from build123d import *

# Parameters (mm, degrees)
SKETCH_1_W             = 88
SKETCH_1_H             = 10
EXTRUDE_1_DEPTH        = 250
SKETCH_2_W             = 2
SKETCH_2_H             = 5
CUT_EXTRUDE_1_DEPTH    = 254.891709199
HOLE_WIZARD_M5_1_D     = 4.2
HOLE_WIZARD_M5_1_DEPTH = 10
HOLE_WIZARD_M5_1_TIP   = 1.2618073
HOLE_WIZARD_M5_2_D     = 4.2
HOLE_WIZARD_M5_2_DEPTH = 10
HOLE_WIZARD_M5_2_TIP   = 1.2618073
SKETCH_7_R             = 3.25
CUT_EXTRUDE_2_DEPTH    = 255.039367028
SKETCH_8_R             = 5.5
CUT_EXTRUDE_3_DEPTH    = 6
SKETCH_9_R             = 2.75
CUT_EXTRUDE_4_DEPTH    = 255.039367028
SKETCH_10_R            = 4.5
CUT_EXTRUDE_5_DEPTH    = 5


with BuildPart() as part:
    # 草图1 → 凸台-拉伸1 (new body)
    with BuildSketch(Plane.XY):
        Rectangle(SKETCH_1_W, SKETCH_1_H)
    extrude(amount=EXTRUDE_1_DEPTH)

    # 草图2 → 切除-拉伸1 (cut, through all)
    with BuildSketch(Plane.XY.offset(250)):
        with Locations((-41, 2.5)):
            Rectangle(SKETCH_2_W, SKETCH_2_H)
        with Locations((41, 2.5)):
            Rectangle(SKETCH_2_W, SKETCH_2_H)
    extrude(amount=-CUT_EXTRUDE_1_DEPTH, mode=Mode.SUBTRACT)

    # M5 螺纹孔1
    with Locations(Plane(origin=(-32, 0, 250), x_dir=(1, 0, 0), z_dir=(0, 0, 1))):
        with Locations((0, 0), (64, 0)):
            Hole(HOLE_WIZARD_M5_1_D / 2, depth=HOLE_WIZARD_M5_1_DEPTH)
            with Locations((0, 0, -(HOLE_WIZARD_M5_1_DEPTH + HOLE_WIZARD_M5_1_TIP / 2))):  # 118° drill point
                Cone(0, HOLE_WIZARD_M5_1_D / 2, HOLE_WIZARD_M5_1_TIP, mode=Mode.SUBTRACT)

    # M5 螺纹孔2
    with Locations(Plane(origin=(32, 0, 0), x_dir=(-1, 0, 0), z_dir=(0, 0, -1))):
        with Locations((0, 0), (64, 0)):
            Hole(HOLE_WIZARD_M5_2_D / 2, depth=HOLE_WIZARD_M5_2_DEPTH)
            with Locations((0, 0, -(HOLE_WIZARD_M5_2_DEPTH + HOLE_WIZARD_M5_2_TIP / 2))):  # 118° drill point
                Cone(0, HOLE_WIZARD_M5_2_D / 2, HOLE_WIZARD_M5_2_TIP, mode=Mode.SUBTRACT)

    # 草图7 → 切除-拉伸2 (cut, through all)
    with BuildSketch(Plane(origin=(0, 5, 0), x_dir=(1, 0, 0), z_dir=(0, 1, 0))):
        with Locations(Location((-15, -80, 0), (0, 0, 270))):
            Circle(SKETCH_7_R)
        with Locations(Location((15, -80, 0), (0, 0, 270))):
            Circle(SKETCH_7_R)
        with Locations(Location((15, -170, 0), (0, 0, 90))):
            Circle(SKETCH_7_R)
        with Locations(Location((-15, -170, 0), (0, 0, 90))):
            Circle(SKETCH_7_R)
    extrude(amount=-CUT_EXTRUDE_2_DEPTH, mode=Mode.SUBTRACT)

    # 草图8 → 切除-拉伸3 (cut)
    with BuildSketch(Plane(origin=(0, 5, 0), x_dir=(1, 0, 0), z_dir=(0, 1, 0))):
        with Locations(Location((-15, -80, 0), (0, 0, 270))):
            Circle(SKETCH_8_R)
        with Locations(Location((15, -80, 0), (0, 0, 270))):
            Circle(SKETCH_8_R)
        with Locations(Location((-15, -170, 0), (0, 0, 270))):
            Circle(SKETCH_8_R)
        with Locations(Location((15, -170, 0), (0, 0, 270))):
            Circle(SKETCH_8_R)
    extrude(amount=-CUT_EXTRUDE_3_DEPTH, mode=Mode.SUBTRACT)

    # 草图9 → 切除-拉伸4 (cut, through all)
    with BuildSketch(Plane.XZ.offset(5)):
        with Locations(Location((-32, 232, 0), (0, 0, 270))):
            Circle(SKETCH_9_R)
        with Locations(Location((-32, 202, 0), (0, 0, 270))):
            Circle(SKETCH_9_R)
    extrude(amount=-CUT_EXTRUDE_4_DEPTH, mode=Mode.SUBTRACT)

    # 草图10 → 切除-拉伸5 (cut)
    with BuildSketch(Plane.XZ.offset(5)):
        with Locations(Location((-32, 232, 0), (0, 0, 270))):
            Circle(SKETCH_10_R)
        with Locations(Location((-32, 202, 0), (0, 0, 270))):
            Circle(SKETCH_10_R)
    extrude(amount=-CUT_EXTRUDE_5_DEPTH, mode=Mode.SUBTRACT)


solid = part.part
Design review of the part built by this model. Coordinates are the model's own, in mm. A direction names the side the tool comes from. Round coordinates to 2 decimals unless told otherwise and drop trailing zeros. Order: outer loops, then holes, each group sorted by start corner. A loop starts at its lowest first (then second) coordinate and runs counter-clockwise, first axis right, second up.
1) Consider section B-B (z = 170). State the section outline as (x, y) points, plus the area to 3 significant figures.
The answers:
outline: (-44, -5) - (-18.25, -5) - (-18.25, -1) - (-20.5, -1) - (-20.5, 5) - (-40, 5) - (-40, 0) - (-42, 0) - (-42, 5) - (-44, 5) - close; (-11.75, -5) - (11.75, -5) - (11.75, -1) - (9.5, -1) - (9.5, 5) - (-9.5, 5) - (-9.5, -1) - (-11.75, -1) - close; (18.25, -5) - (44, -5) - (44, 5) - (42, 5) - (42, 0) - (40, 0) - (40, 5) - (20.5, 5) - (20.5, -1) - (18.25, -1) - close
area: 676 mm2
2) Draft analysis for pull direction Z (two halves, no side actions). For faces 1 (the conical face through (31.8, 0.31, 11.04)), 2 (the flat face through (-35, 0, 202)), 3 (the flat face through (-44, 0, 123)), state which applies: released by +Z, released by -Z, zero draft, split by the parting line, or undercut.
The answers:
face 1: released by -Z
face 2: undercut
face 3: zero draft
3) Clearance check with flat-ended pins moving along their axes: pin 1 Ø9 at (x, z) = (15, 79.5) entering from +Y; pin 2 Ø7 at (x, z) = (-32, 232) entering from -Y; pin 3 Ø4 at (x, y) = (-32, 0) entering from -Z. State where each tip first meets the part, or that it passes through.
The answers:
pin 1: stops at y = -1
pin 2: stops at y = 0
pin 3: stops at z = 10.06
4) Consider section A-A (x = -15). State the section outline as (y, z) points, plus the area to 3 significant figures.
The answers:
outline: (-5, 0) - (5, 0) - (5, 74.5) - (-1, 74.5) - (-1, 76.75) - (-5, 76.75) - close; (-5, 83.25) - (-1, 83.25) - (-1, 85.5) - (5, 85.5) - (5, 164.5) - (-1, 164.5) - (-1, 166.75) - (-5, 166.75) - close; (-5, 173.25) - (-1, 173.25) - (-1, 175.5) - (5, 175.5) - (5, 250) - (-5, 250) - close
area: 2,320 mm2
5) For L1, parallel to X at y = -4.2, z = 80; L2, parallel to X at y = 4.5, z = 26; L3, parallel to X at y = 0.45, z = 80, list the stretches that pass through material, from the lowest coordinate up.
The answers:
L1: x = -44 to -18.25, -11.75 to 11.75, 18.25 to 44
L2: x = -44 to -42, -40 to 40, 42 to 44
L3: x = -44 to -42, -40 to -20.5, -9.5 to 9.5, 20.5 to 40, 42 to 44
6) Consider section C-C (z = 69.5). State the section outline as (x, y) points, plus the area to 3 significant figures.
The answers:
outline: (-44, -5) - (44, -5) - (44, 5) - (42, 5) - (42, 0) - (40, 0) - (40, 5) - (-40, 5) - (-40, 0) - (-42, 0) - (-42, 5) - (-44, 5) - close
area: 860 mm2
7) Machinability: for faces 4 (the cylindrical face through (-33.72, -2.54, 227.84)), 5 (the cylindrical face through (-14.758, 2.042, 164.505)), 6 (the cylindrical face through (34.1, 0.09, 244.93)), which of the approach directions +Z, -Z, +X, -X, +Y, -Y give a long, thin tool a straight path to every point of the face, cutting with its end or side? Answer none if there is none.
The answers:
face 4: -Y
face 5: +Y
face 6: +Z
